from build123d import *

# Parameters (mm, degrees)
SKETCH1_R             = 100
SKETCH1_R_2           = 75
BOSS_EXTRUDE1_DEPTH   = 20
BOSS_EXTRUDE2_START   = 80
SKETCH2_R             = 15
BOSS_EXTRUDE2_DEPTH   = 70
M6_TAPPED_HOLE1_D     = 5
M6_TAPPED_HOLE1_DEPTH = 17
M6_TAPPED_HOLE1_TIP   = 1.502151548


with BuildPart() as part:
    # Sketch1 → Boss-Extrude1 (new body)
    with BuildSketch(Plane(origin=(0, 0, 0), x_dir=(1, 0, 0), z_dir=(0, 1, 0))):
        with Locations(Location((0, 0, 0), (0, 0, 270))):
            Circle(SKETCH1_R)
        with Locations(Location((0, 0, 0), (0, 0, 270))):
            Circle(SKETCH1_R_2, mode=Mode.SUBTRACT)
    extrude(amount=BOSS_EXTRUDE1_DEPTH)

    # Sketch2 → Boss-Extrude2 (add)
    with BuildSketch(Plane(origin=(0, 0, 0), x_dir=(0, 0, -1), z_dir=(1, 0, 0)).offset(BOSS_EXTRUDE2_START)):
        with Locations(Location((0, 10, 0), (0, 0, 138.189685104))):
            Circle(SKETCH2_R)
    extrude(amount=BOSS_EXTRUDE2_DEPTH)

    # M6 Tapped Hole1
    with Locations(Plane(origin=(150, 0, 0), x_dir=(0, 0, -1), z_dir=(1, 0, 0))):
        with Locations((0, 10)):
            Hole(M6_TAPPED_HOLE1_D / 2, depth=M6_TAPPED_HOLE1_DEPTH)
            with Locations((0, 0, -(M6_TAPPED_HOLE1_DEPTH + M6_TAPPED_HOLE1_TIP / 2))):  # 118° drill point
                Cone(0, M6_TAPPED_HOLE1_D / 2, M6_TAPPED_HOLE1_TIP, mode=Mode.SUBTRACT)


solid = part.part
Can you work these out from the model? Positions are in its coordinate system, mm. A direction names the side the tool comes from. Give positions to 0.01 mm unless a question says otherwise; leave off trailing zeros. Loops run counter-clockwise (first coordinate to the right, second up) from the corner with the lowest first, then second, coordinate; pieces in that order, holes last. Notation, with made-up numbers: (8, 16) -> (29, 16) arc R33 cw to (29, 45) -> close; hole circle Ø10 at (-27.75, 3.5). An arc over 180 degrees is marked (long way). Write item = value, one per line.
1) Suppose I cut it at B-B on z = 52. Write out the boundary of the cut face in (x, y), then the cut area to 3 significant figures.
Check result:
outline = (-85.42, 0) -> (-54.05, 0) -> (-54.05, 20) -> (-85.42, 20) -> close; (54.05, 0) -> (85.42, 0) -> (85.42, 20) -> (54.05, 20) -> close
area = 1,250 mm2
2) I need wall thicknesses on L1, parallel to Z at x = 144, y = 10; L2, parallel to Y at x = 137, z = 0; L3, parallel to X at y = 13, z = -41. Which ranges of each line are inside material? Lowest first, please. Write a range as from..to.
Check result:
L1 = -15..-2.5, 2.5..15
L2 = -5..7.5, 12.5..25
L3 = -91.21..-62.8, 62.8..91.21
3) Suppose I cut it at A-A on x = 0. Write out the boundary of the cut face in (y, z), then the cut area to 3 significant figures.
Check result:
outline = (0, -100) -> (20, -100) -> (20, -75) -> (0, -75) -> close; (0, 75) -> (20, 75) -> (20, 100) -> (0, 100) -> close
area = 1,000 mm2
4) Thinking about a two-plate mould opening in Y: for faces 4 (the flat face through (74, 0, 14)), 5 (the cylindrical face through (141.38, 7.56, -0.54)), 6 (the conical face through (131.76, 10.37, -0.23)), 7 (the flat face through (80, 22, -1)), which applies, released by +Y, released by -Y, zero draft, split by the parting line, or undercut?
Check result:
face_4 = released by -Y
face_5 = undercut
face_6 = undercut
face_7 = zero draft
5) For faces 1 (the flat face through (80, -1, -1)), 2 (the cylindrical face through (114.51, -4.927, -1.482)), 3 (the cylindrical face through (-45.636, 9.86, -59.517)), which set-ups out of +Z, -Z, +X, -X, +Y, -Y let a thin tool reach every point of the face, with its end or its side?
Check result:
face_1 = +Z, -Z, -X, -Y
face_2 = +X
face_3 = +Y, -Y
6) Suppose I cut it at C-C on y = 15.5. Write out the boundary of the cut face in (x, z), then the cut area to 3 significant figures.
Check result:
outline = (99.02, -13.96) -> (150, -13.96) -> (150, 13.96) -> (99.02, 13.96) arc R100 ccw (long way) to start; hole circle Ø150 at (0, 0)
area = 15,100 mm2
7) Will these pins go through, and if not, where does the flat tip stop? pin 1 (4 mm diameter, centred on y = 22.5, z = -4, fed in from -X); pin 2 (12 mm diameter, centred on y = 7.5, z = 55, fed in from -X); pin 3 (6 mm diameter, centred on x = -63.5, z = -61, fed in from +Y).
Check result:
pin_1 = 80
pin_2 = -87.17
pin_3 = 20
